```python
from build123d import *

# Parameters (mm, degrees)
HOLE_WIZARD_1_D           = 11
HOLE_WIZARD_1_CBORE_D     = 18
HOLE_WIZARD_1_CBORE_DEPTH = 11
PATTERN_CIRCULAR_1_COUNT  = 6
CHAMFER_1_SIZE            = 0.5


with BuildPart() as part:
    # 草图1 → 旋转1 (revolve)
    with BuildSketch(Plane(origin=(0, 0, 0), x_dir=(1, 0, 0), z_dir=(0, 1, 0))):
        Polygon((-34, 0), (-67.5, 0), (-67.5, 20), (-42.5, 20), (-42.5, 33), (-34, 33), align=None)
    revolve(axis=Axis((0, 0, 0), (0, 0, 1)))

    # 打孔尺寸(%根据)内六角圆柱头螺钉的类型1 (through all)
    with Locations(Plane.XY):
        with Locations((55, 0)):
            hole_wizard_1 = CounterBoreHole(HOLE_WIZARD_1_D / 2, HOLE_WIZARD_1_CBORE_D / 2, HOLE_WIZARD_1_CBORE_DEPTH)

    # 阵列(圆周)1: 打孔尺寸(%根据)内六角圆柱头螺钉的类型1 ×6 about axis
    pattern_circular_1_axis = Axis((0, 0, 0), (0, 0, 1))
    for i in range(1, PATTERN_CIRCULAR_1_COUNT):
        add(hole_wizard_1.rotate(pattern_circular_1_axis, i * 360 / PATTERN_CIRCULAR_1_COUNT), mode=Mode.SUBTRACT)

    # 倒角1
    chamfer_1_edges = [part.edges().sort_by_distance(p)[0] for p in [
        (67.5, 0, 0),
        (34, 0, 0),
        (34, 0, -33),
        (42.5, 0, -33),
        (67.5, 0, -20),
    ]]
    chamfer(chamfer_1_edges, length=CHAMFER_1_SIZE)


solid = part.part
```
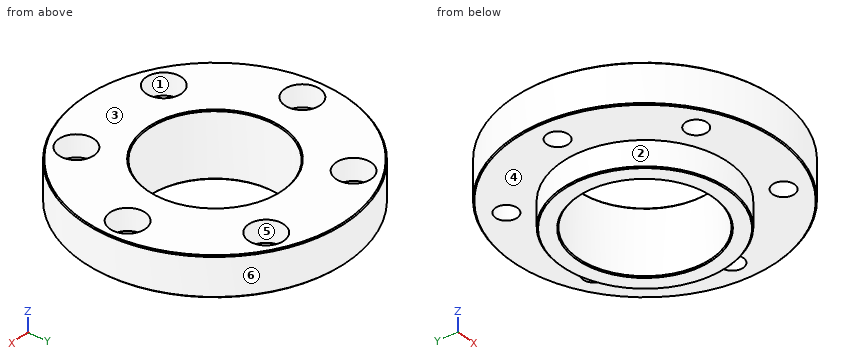
Work out the finished part from the listing and answer in its coordinate system (mm). Face numbers are marked on the shaded views. A direction names the side the tool comes from. Give positions to 0.01 mm unless a question says otherwise; leave off trailing zeros. Write each loop counter-clockwise with the first axis right and the second up, starting at its lowest first coordinate (ties: lowest second). Pieces come first, ordered by that corner, then holes.
(1) The part is cut by section C-C on z = -9. Write down the section's boundary in (x, y).
Final values:
outline: circle Ø135 at (0, 0); hole circle Ø18 at (-55, 0); hole circle Ø18 at (-27.5, -47.63); hole circle Ø18 at (-27.5, 47.63); hole circle Ø68 at (0, 0); hole circle Ø18 at (27.5, -47.63); hole circle Ø18 at (27.5, 47.63); hole circle Ø18 at (55, 0)
(2) Flat-ended cylindrical pins translate along their axes: pin 1 Ø8 at (x, z) = (24, -13) entering from -Y; pin 2 Ø14.5 at (x, y) = (-55, 0) entering from +Z; pin 3 Ø23.5 at (x, y) = (27.5, -47.63) entering from -Z; pin 4 Ø10 at (x, y) = (55, 0) entering from +Z. Find the tip coordinate at first contact, or state that the pin passes through.
Final values:
pin 1: stops at y = -64.47
pin 2: stops at z = -11
pin 3: stops at z = -20
pin 4: passes through
(3) The mould has two halves that part along X. Classify the marked faces 4, 5 and 6: pulls with the +X half, pulls with the -X half, needs draft (parallel to the pull), parting line crosses it, or undercut.
Final values:
face 4: needs draft
face 5: undercut
face 6: parting line crosses it
(4) Straight lines are drawn through the part: line 1 (Y direction, x = 28.5, z = -12); line 2 (Y direction, x = 1, z = -28); line 3 (Y direction, x = 55, z = -6.5). For each, find the intervals that lie inside material, in ascending order.
Final values:
line 1: y = -61.19 to -53.04, -42.22 to -18.54, 18.54 to 42.22, 53.04 to 61.19
line 2: y = -42.49 to -33.99, 33.99 to 42.49
line 3: y = -39.13 to -9, 9 to 39.13
(5) The part is cut by section A-A on z = -26. Write down the section's boundary in (x, y), plus the area to 3 significant figures.
Final values:
outline: circle Ø85 at (0, 0); hole circle Ø68 at (0, 0)
area: 2,040 mm2
(6) The part is cut by section B-B on y = 0. Count the separate pieces of the cut face and the enclosed holes in it, plus the area to 3 significant figures.
Final values:
separate pieces: 4
enclosed holes: 0
area: 966 mm2
(7) Which of the six approach directions +Z, -Z, +X, -X, +Y, -Y give full straight-line access (tool end or side, diameter ignored) to the marked faces 1, 2 and 3?
Final values:
face 1: +Z
face 2: -Z
face 3: +Z, +X, -X, +Y, -Y
